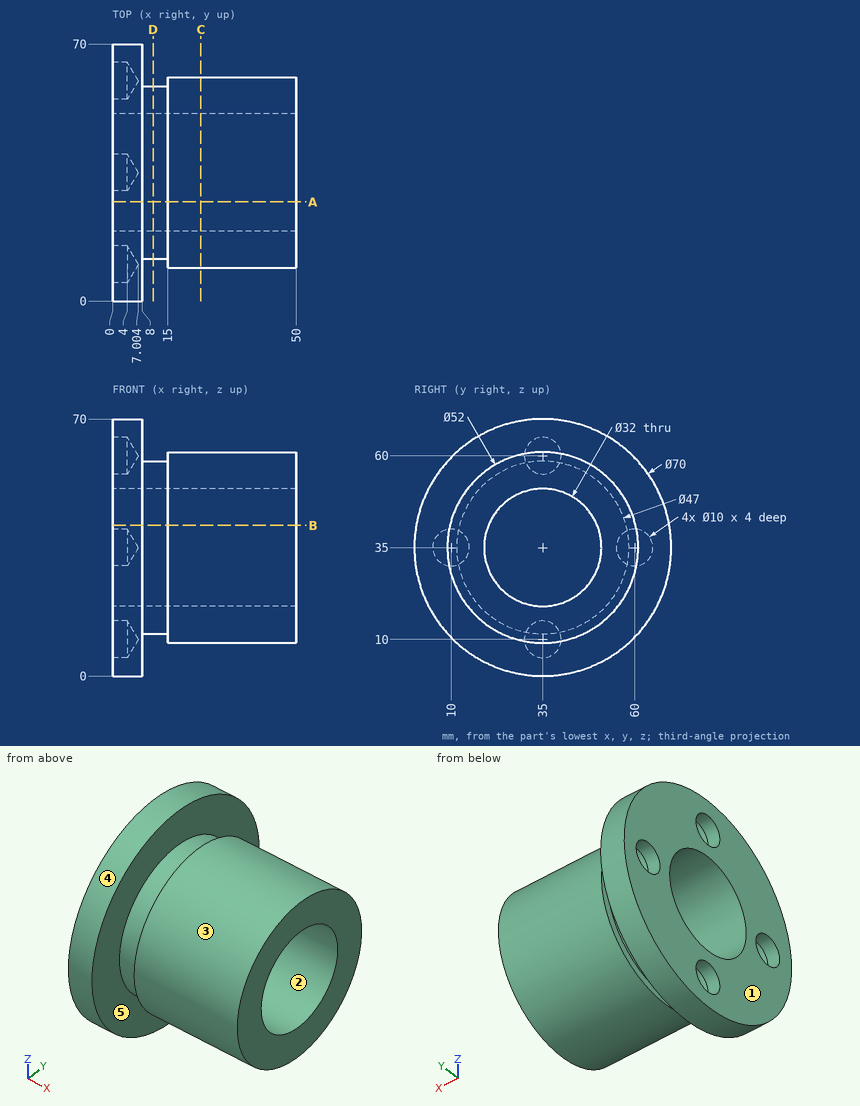
Design review of the part shown in the three views and the two pictorial views. Dimensions are in mm from the part's minimum x, y and z. A direction names the side the tool comes from. Round coordinates to 2 decimals unless told otherwise and drop trailing zeros. Order: outer loops, then holes, each group sorted by start corner. A loop starts at its lowest first (then second) coordinate and runs counter-clockwise, first axis right, second up. Notation, with made-up numbers: (31.5, 88) - (70.5, 88) arc R27 ccw to (70.5, 115) - close; hole circle Ø11 at (69, 5.5). An arc over 180 degrees is marked (long way). One line per question, with ' | ' between items.
Item 1: Take a section at B-B, the plane z = 41. Write out the cut boundary in (x, y), then the cut area to 3 significant figures.
Checks:
outline: (0, 0.52) - (8, 0.52) - (8, 12.28) - (15, 12.28) - (15, 9.7) - (50, 9.7) - (50, 20.17) - (0, 20.17) - close; (0, 49.83) - (50, 49.83) - (50, 60.3) - (15, 60.3) - (15, 57.72) - (8, 57.72) - (8, 69.48) - (0, 69.48) - close | area: 1,160 mm²
Item 2: Machinability: for the marked faces 4 and 5, which of the approach directions +Z, -Z, +X, -X, +Y, -Y give a long, thin tool a straight path to every point of the face, cutting with its end or side? Answer none if there is none.
Checks:
face 4: +X, -X | face 5: none
Item 3: Draft analysis for pull direction Z (two halves, no side actions). For the marked faces 1, 2 and 3, state which applies: +Z half, -Z half, draft (parallel to the pull), parting line (faces both ways), or undercut.
Checks:
face 1: draft | face 2: undercut | face 3: parting line
Item 4: Take a section at C-C, the plane x = 24. Write out the cut boundary in (y, z).
Checks:
outline: circle Ø52 at (35, 35); hole circle Ø32 at (35, 35)
Item 5: Take a section at A-A, the plane y = 27. Write out the cut boundary in (x, z).
Checks:
outline: (0, 0.93) - (8, 0.93) - (8, 12.9) - (15, 12.9) - (15, 10.26) - (50, 10.26) - (50, 21.14) - (0, 21.14) - close; (0, 48.86) - (50, 48.86) - (50, 59.74) - (15, 59.74) - (15, 57.1) - (8, 57.1) - (8, 69.07) - (0, 69.07) - close
Item 6: For P1, Ø3, axis at x = 43, z = 43, coming from the +Y side; P2, Ø4, axis at x = 9.5, y = 48, coming from the +Z side (1 decimal); P3, Ø8, axis at x = 23.5, y = 29, coming from the -Z side; P4, Ø10, axis at y = 51.5, z = 57, coming from the +X side, all flat-tipped, find the tip position at first contact; note any pin that passes through.
Checks:
P1: y = 60.17 | P2: z = 68 | P3: z = 9.08 | P4: x = 50
Item 7: Wall thickness on line 1 (Y direction, x = 2, z = 35); line 2 (Z direction, x = 17, y = 35); line 3 (X direction, y = 59.5, z = 42): over which ranges is each line inside the solid? List them lowest first. Write a range as [from, to].
Checks:
line 1: [0, 5], [15, 19], [51, 55], [65, 70] | line 2: [9, 19], [51, 61] | line 3: [0, 8], [15, 50]
Item 8: Take a section at D-D, the plane x = 11. Write out the cut boundary in (y, z), then the cut area to 3 significant figures.
Checks:
outline: circle Ø47 at (35, 35); hole circle Ø32 at (35, 35) | area: 931 mm²
